Answer from the drawing. Dimensions are ordinates in mm from the lowest x, y and z of the part. A direction names the side the tool comes from. Coordinates: 2 decimals unless noted, no trailing zeros. Loops run counter-clockwise (first coordinate to the right, second up) from the corner with the lowest first, then second, coordinate; pieces in that order, holes last. Notation, with made-up numbers: (49.25, -10) -> (84.25, -10) arc R11 ccw to (84.25, -2) -> close; hole circle Ø7 at (10.25, 1). An arc over 180 degrees is marked (long way). Answer as CSV lines item,"result".
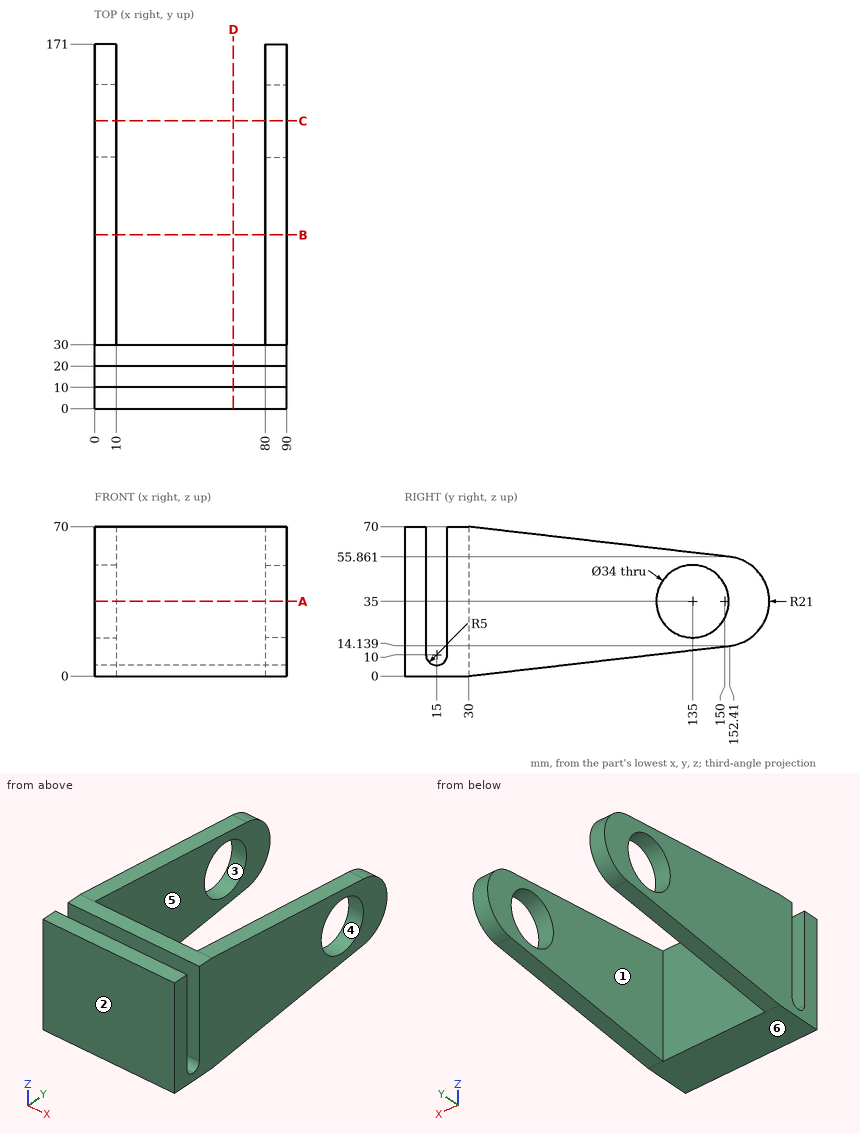
(1) A cutting plane is placed at B-B, the plane y = 81.5. Write down the section's boundary in (x, z), and give its area (3 significant figures).
Computed values:
outline,"(0, 5.95) -> (10, 5.95) -> (10, 64.05) -> (0, 64.05) -> close; (80, 5.95) -> (90, 5.95) -> (90, 64.05) -> (80, 64.05) -> close"
area,"1,160 mm2"
(2) Consider line 1 along Y through (x, z) = (82, 35); line 2 along X through (y, z) = (82.5, 57); line 3 along Y through (x, z) = (30.5, 37.5). Determine where each line is inside the solid, lowest interval first.
Computed values:
line 1,"0 to 10, 20 to 118, 152 to 171"
line 2,"0 to 10, 80 to 90"
line 3,"0 to 10, 20 to 30"
(3) A cutting plane is placed at D-D, the plane x = 65. Write down the section's boundary in (y, z), and give its area (3 significant figures).
Computed values:
outline,"(0, 0) -> (30, 0) -> (30, 70) -> (20, 70) -> (20, 10) arc R5 cw to (10, 10) -> (10, 70) -> (0, 70) -> close"
area,"1,460 mm2"
(4) A flat-ended cylindrical pin translates along its axis: pin 1 Ø2 at (x, z) = (57.5, 62.5) entering from +Y. Find the tip coordinate at first contact, or state that the pin passes through.
Computed values:
pin 1,"y = 30"
(5) A cutting plane is placed at A-A, the plane z = 35. Write down the section's boundary in (x, y).
Computed values:
outline,"(0, 0) -> (90, 0) -> (90, 10) -> (0, 10) -> close; (0, 20) -> (90, 20) -> (90, 118) -> (80, 118) -> (80, 30) -> (10, 30) -> (10, 118) -> (0, 118) -> close; (0, 152) -> (10, 152) -> (10, 171) -> (0, 171) -> close; (80, 152) -> (90, 152) -> (90, 171) -> (80, 171) -> close"
(6) For a pull along Y with two mould halves and no side action, classify the marked faces 1, 2, 3 and 4 as pulls with the +Y half, pulls with the -Y half, needs draft (parallel to the pull), parting line crosses it, or undercut.
Computed values:
face 1,"needs draft"
face 2,"pulls with the -Y half"
face 3,"undercut"
face 4,"undercut"
(7) Which of the six approach directions +Z, -Z, +X, -X, +Y, -Y give full straight-line access (tool end or side, diameter ignored) to the marked faces 5 and 6?
Computed values:
face 5,"+Z, -Z, +Y"
face 6,"-Z, +X, -X, +Y, -Y"
(8) A cutting plane is placed at C-C, the plane y = 135. Write down the section's boundary in (x, z), and give its area (3 significant figures).
Computed values:
outline,"(0, 12.13) -> (10, 12.13) -> (10, 18) -> (0, 18) -> close; (0, 52) -> (10, 52) -> (10, 57.87) -> (0, 57.87) -> close; (80, 12.13) -> (90, 12.13) -> (90, 18) -> (80, 18) -> close; (80, 52) -> (90, 52) -> (90, 57.87) -> (80, 57.87) -> close"
area,"235 mm2"
